Answer from the drawing. Dimensions are ordinates in mm from the lowest x, y and z of the part. Give positions to 0.01 mm unless a question says otherwise; leave off trailing zeros. Loops run counter-clockwise (first coordinate to the right, second up) from the corner with the lowest first, then second, coordinate; pieces in that order, holes last. Notation, with made-up numbers: (-1.75, 38) - (10.25, 38) arc R18 ccw to (10.25, 55) - close; hole circle Ø6 at (71, -24.5). An arc over 180 degrees is marked (long way). Put each result on its own line as item: value. Start each with the question number.
1. A cutting plane is placed at C-C, the plane z = 6.5. Determine the outline of the cut face in (x, y), plus the area to 3 significant figures.
2. A cutting plane is placed at B-B, the plane x = 12.5. Determine the outline of the cut face in (y, z), plus the area to 3 significant figures.
3. Consider L1, parallel to Y at x = 12.5, z = 5.5; L2, parallel to X at y = 17, z = 9.75; L3, parallel to X at y = 19.5, z = 3.25. Determine where each line is inside the solid, lowest interval first. Write a range as from..to.
4. A cutting plane is placed at A-A, the plane y = 102.5. Determine the outline of the cut face in (x, z).
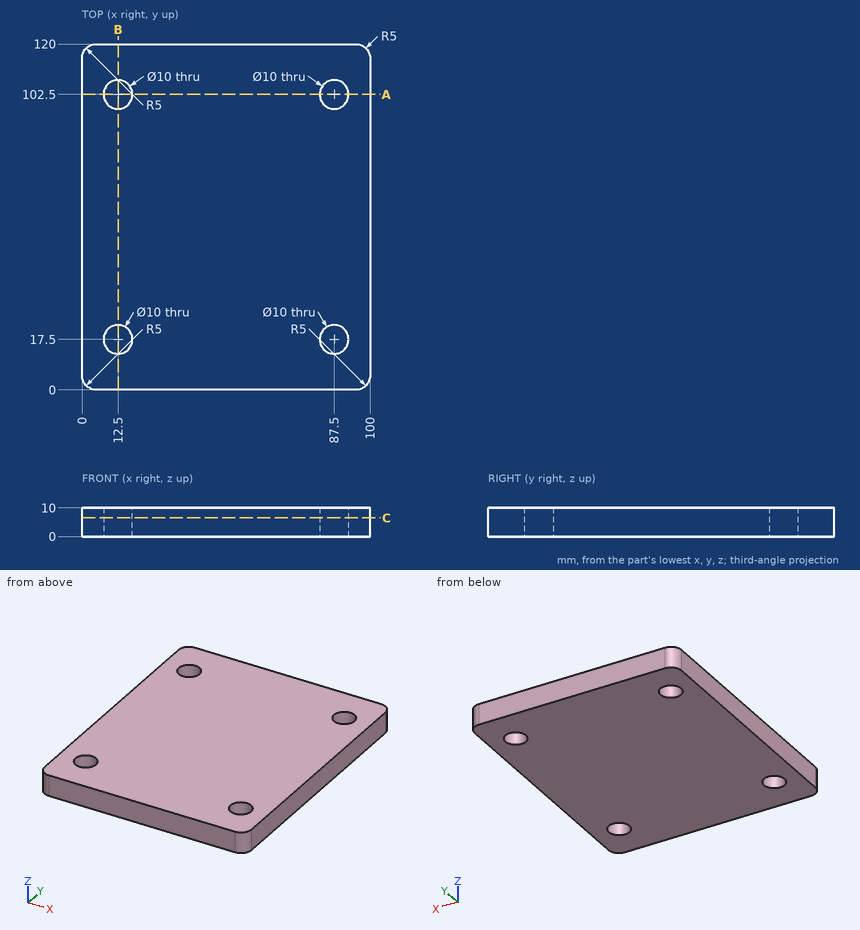
Return value:
1. outline: (0, 5) arc R5 ccw to (5, 0) - (95, 0) arc R5 ccw to (100, 5) - (100, 115) arc R5 ccw to (95, 120) - (5, 120) arc R5 ccw to (0, 115) - close; hole circle Ø10 at (12.5, 17.5); hole circle Ø10 at (12.5, 102.5); hole circle Ø10 at (87.5, 17.5); hole circle Ø10 at (87.5, 102.5)
1. area: 11,700 mm2
2. outline: (0, 0) - (12.5, 0) - (12.5, 10) - (0, 10) - close; (22.5, 0) - (97.5, 0) - (97.5, 10) - (22.5, 10) - close; (107.5, 0) - (120, 0) - (120, 10) - (107.5, 10) - close
2. area: 1,000 mm2
3. L1: y = 0..12.5, 22.5..97.5, 107.5..120
3. L2: x = 0..7.53, 17.47..82.53, 92.47..100
3. L3: x = 0..7.92, 17.08..82.92, 92.08..100
4. outline: (0, 0) - (7.5, 0) - (7.5, 10) - (0, 10) - close; (17.5, 0) - (82.5, 0) - (82.5, 10) - (17.5, 10) - close; (92.5, 0) - (100, 0) - (100, 10) - (92.5, 10) - close
